```python
from build123d import *

# Parameters (mm, degrees)
SKETCH_1_W                = 210
SKETCH_1_H                = 90
EXTRUDE_1_DEPTH           = 10
CHAMFER_1_SIZE            = 3
HOLE_WIZARD_2_D           = 5.5
HOLE_WIZARD_2_DEPTH       = 10.1
HOLE_WIZARD_2_CBORE_D     = 10
HOLE_WIZARD_2_CBORE_DEPTH = 5.7
HOLE_WIZARD_2_TIP         = 1.652366702
SKETCH_4_W                = 100
SKETCH_4_H                = 22.5
CUT_EXTRUDE_1_DEPTH       = 20
CHAMFER_2_SIZE            = 3
FILLET_1_R                = 5
HOLE_WIZARD_0_D           = 4.5
HOLE_WIZARD_0_DEPTH       = 25
HOLE_WIZARD_0_CBORE_D     = 8
HOLE_WIZARD_0_CBORE_DEPTH = 4.6
HOLE_WIZARD_0_TIP         = 1.351936393
MM_0_D                    = 4
MM_0_DEPTH                = 25
MM_0_TIP                  = 1.201721238
HOLE_WIZARD_M5_1_D        = 4.2
HOLE_WIZARD_M5_1_DEPTH    = 12.4
HOLE_WIZARD_M5_1_TIP      = 1.2618073


with BuildPart() as part:
    # 草图1 → 凸台-拉伸1 (new body)
    with BuildSketch(Plane(origin=(0, 0, 0), x_dir=(1, 0, 0), z_dir=(0, 1, 0))):
        Rectangle(SKETCH_1_W, SKETCH_1_H)
    extrude(amount=EXTRUDE_1_DEPTH)

    # 倒角1
    chamfer_1_edges = [part.edges().sort_by_distance(p)[0] for p in [
        (105, 5, 45),
        (-105, 5, 45),
        (-105, 5, -45),
        (105, 5, -45),
    ]]
    chamfer(chamfer_1_edges, length=CHAMFER_1_SIZE)

    # 打孔尺寸(%根据)内六角圆柱头螺钉的类型2
    with Locations(Plane(origin=(0, 10, 0), x_dir=(1, 0, 0), z_dir=(0, 1, 0))):
        with Locations((58, -37), (58, 37), (88, 37), (88, -37)):
            CounterBoreHole(HOLE_WIZARD_2_D / 2, HOLE_WIZARD_2_CBORE_D / 2, HOLE_WIZARD_2_CBORE_DEPTH, depth=HOLE_WIZARD_2_DEPTH)
            with Locations((0, 0, -(HOLE_WIZARD_2_DEPTH + HOLE_WIZARD_2_TIP / 2))):  # 118° drill point
                Cone(0, HOLE_WIZARD_2_D / 2, HOLE_WIZARD_2_TIP, mode=Mode.SUBTRACT)

    # 草图4 → 切除-拉伸1 (cut)
    with BuildSketch(Plane(origin=(0, 10, 0), x_dir=(1, 0, 0), z_dir=(0, 1, 0))):
        with Locations((-55, -33.75)):
            Rectangle(SKETCH_4_W, SKETCH_4_H)
        with Locations((-55, 33.75)):
            Rectangle(SKETCH_4_W, SKETCH_4_H)
    extrude(amount=-CUT_EXTRUDE_1_DEPTH, mode=Mode.SUBTRACT)

    # 倒角2
    chamfer_2_edges = [part.edges().sort_by_distance(p)[0] for p in [
        (-105, 5, 22.5),
        (-5, 5, 45),
        (-5, 5, -45),
        (-105, 5, -22.5),
    ]]
    chamfer(chamfer_2_edges, length=CHAMFER_2_SIZE)

    # 圆角1
    fillet_1_edges = [part.edges().sort_by_distance(p)[0] for p in [
        (-5, 5, 22.5),
        (-5, 5, -22.5),
    ]]
    fillet(fillet_1_edges, radius=FILLET_1_R)

    # 打孔尺寸(%根据)内六角圆柱头螺钉的类型0
    with Locations(Plane(origin=(0, 0, 0), x_dir=(-1, 0, 0), z_dir=(0, -1, 0))):
        with Locations((21.3, 10.3), (21.3, -9.7), (1.3, 10.3), (1.3, -9.7)):
            CounterBoreHole(HOLE_WIZARD_0_D / 2, HOLE_WIZARD_0_CBORE_D / 2, HOLE_WIZARD_0_CBORE_DEPTH, depth=HOLE_WIZARD_0_DEPTH)
            with Locations((0, 0, -(HOLE_WIZARD_0_DEPTH + HOLE_WIZARD_0_TIP / 2))):  # 118° drill point
                Cone(0, HOLE_WIZARD_0_D / 2, HOLE_WIZARD_0_TIP, mode=Mode.SUBTRACT)

    # 大小mm 暗销孔0
    with Locations(Plane(origin=(0, 0, 0), x_dir=(-1, 0, 0), z_dir=(0, -1, 0))):
        with Locations((11.3, -9.7), (11.3, 10.231708661)):
            Hole(MM_0_D / 2, depth=MM_0_DEPTH)
            with Locations((0, 0, -(MM_0_DEPTH + MM_0_TIP / 2))):  # 118° drill point
                Cone(0, MM_0_D / 2, MM_0_TIP, mode=Mode.SUBTRACT)

    # M5 螺纹孔1
    with Locations(Plane(origin=(0, 10, 0), x_dir=(1, 0, 0), z_dir=(0, 1, 0))):
        with Locations((97, -22.5), (97, 0), (97, 22.5)):
            Hole(HOLE_WIZARD_M5_1_D / 2, depth=HOLE_WIZARD_M5_1_DEPTH)
            with Locations((0, 0, -(HOLE_WIZARD_M5_1_DEPTH + HOLE_WIZARD_M5_1_TIP / 2))):  # 118° drill point
                Cone(0, HOLE_WIZARD_M5_1_D / 2, HOLE_WIZARD_M5_1_TIP, mode=Mode.SUBTRACT)


solid = part.part
```
Geometry: final body of the model. Coordinates: model frame, mm. A direction names the side the tool comes from. Coordinates: 2 decimals unless noted, no trailing zeros. Order: outer loops, then holes, each group sorted by start corner. A loop starts at its lowest first (then second) coordinate and runs counter-clockwise, first axis right, second up. Notation, with made-up numbers: M 83,50 L 108,50 A24 ccw 108,86 Z; hole C -38,-30.75 d1. An arc over 180 degrees is marked long. Answer in a Markdown table with one row per item. Add a question column.
Q1. Section query B-B on z = -37. Return the cut outline in (x, y), and give its area (3 significant figures).
Q2. Section query D-D on y = 7. Count the separate pieces of the cut face and the enclosed holes in it, and give its area (3 significant figures).
Q3. Section query C-C on x = 97. Return the cut outline in (y, z).
Q4. Contact query for flat-ended pins moving along their axis: P1, Ø3, axis at x = -42, y = 6, coming from the -Z side; P2, Ø1, axis at x = -74.5, y = 5, coming from the +Z side; P3, Ø4.5, axis at x = -11.3, z = -10.23, coming from the -Y side; P4, Ø6, axis at y = 6.5, z = 26, coming from the -X side. Output: stop coordinate, or through.
Q5. Line query: L1, parallel to Z at x = -21.3, y = 7.95; L2, parallel to Z at x = 97, y = 7.5; L3, parallel to Z at x = 58, y = 6.85. Output: solid intervals per line, ascending.
Q6. Section query A-A on x = 58. Return the cut outline in (y, z).
Q7. Mould query, pull axis Z, two halves, no side actions, for faces 1 (the flat face through (105, 5, 1)), 2 (the flat face through (49, 5, 45)), 3 (the cylindrical face through (99.1, 4.93, -0.09)). Classes: released by +Z, released by -Z, zero draft, split by the parting line, or undercut.
Q8. Reachability of faces 4 (the flat face through (-3, 4.6, -8.6)), 5 (the cylindrical face through (57.349, 7.19, -41.957)), 6 (the flat face through (-5, 5, -35)) from +Z, -Z, +X, -X, +Y, -Y: full face, straight path, thin tool, end or side. Return the list, or none.
Completed:
| question | item | result |
|---|---|---|
| 1 | outline | M -5,0 L 55.25,0 L 55.25,4.3 L 53,4.3 L 53,10 L -5,10 Z; M 60.75,0 L 85.25,0 L 85.25,4.3 L 83,4.3 L 83,10 L 63,10 L 63,4.3 L 60.75,4.3 Z; M 90.75,0 L 105,0 L 105,10 L 93,10 L 93,4.3 L 90.75,4.3 Z |
| 1 | area | 939 mm2 |
| 2 | separate pieces | 1 |
| 2 | enclosed holes | 13 |
| 2 | area | 13,900 mm2 |
| 3 | outline | M 0,-45 L 10,-45 L 10,-24.6 L 0,-24.6 Z; M 0,-20.4 L 10,-20.4 L 10,-2.1 L 0,-2.1 Z; M 0,2.1 L 10,2.1 L 10,20.4 L 0,20.4 Z; M 0,24.6 L 10,24.6 L 10,45 L 0,45 Z |
| 4 | P1 | stops at z = -22.5 |
| 4 | P2 | stops at z = 22.5 |
| 4 | P3 | stops at y = 0 |
| 4 | P4 | stops at x = -7.82 |
| 5 | L1 | z = -22.5 to -12.55, -8.05 to 7.45, 11.95 to 22.5 |
| 5 | L2 | z = -45 to -24.6, -20.4 to -2.1, 2.1 to 20.4, 24.6 to 45 |
| 5 | L3 | z = -45 to -42, -32 to 32, 42 to 45 |
| 6 | outline | M 0,-45 L 10,-45 L 10,-42 L 4.3,-42 L 4.3,-39.75 L 0,-39.75 Z; M 0,-34.25 L 4.3,-34.25 L 4.3,-32 L 10,-32 L 10,32 L 4.3,32 L 4.3,34.25 L 0,34.25 Z; M 0,39.75 L 4.3,39.75 L 4.3,42 L 10,42 L 10,45 L 0,45 Z |
| 7 | face 1 | zero draft |
| 7 | face 2 | released by +Z |
| 7 | face 3 | undercut |
| 8 | face 4 | -Y |
| 8 | face 5 | +Y |
| 8 | face 6 | -Z, -X, +Y, -Y |
